Input: dimensioned drawing with shaded views. Units: mm. Origin: part minimum x, y, z. A direction names the side the tool comes from. Coordinates: 2 decimals unless noted, no trailing zeros. Order: outer loops, then holes, each group sorted by start corner. A loop starts at its lowest first (then second) coordinate and runs counter-clockwise, first axis right, second up.
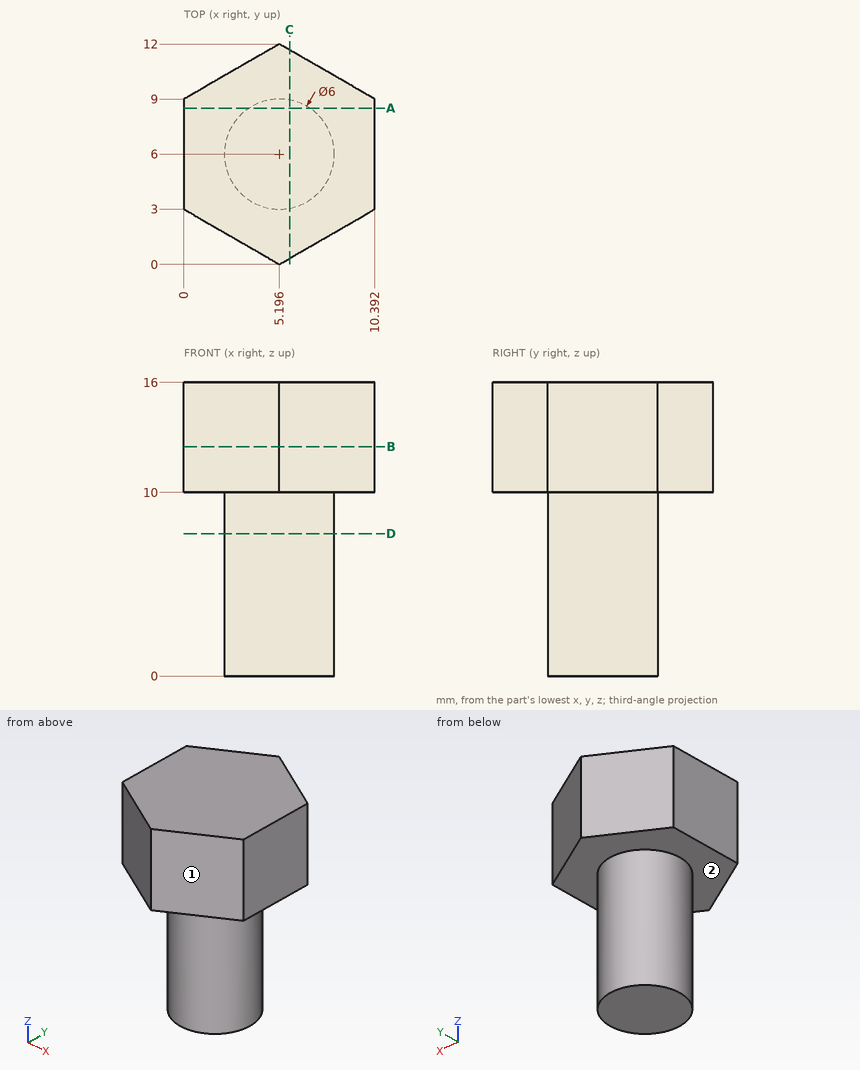
1. Contact query for flat-ended pins moving along their axis: P1, Ø5, axis at x = 9, z = 13.5, coming from the +Y side; P2, Ø4, axis at x = 2.5, z = 7.5, coming from the +Y side. Output: stop coordinate, or through.
2. Section query C-C, the plane x = 5.75. Output: boundary loops of the cut face in (y, z).
3. Access query for the marked faces 1 and 2. Directions: +Z, -Z, +X, -X, +Y, -Y. A direction counts if a zero-diameter tool reaches every point of the face in a straight line with its end or side. Return the directions, or none.
4. Section query D-D, the plane z = 7.75. Output: boundary loops of the cut face in (x, y), plus the area to 3 significant figures.
5. Material intervals for line 1 along Z through (x, y) = (10.25, 5.25); line 2 along Y through (x, z) = (7.5, 0.5); line 3 along Y through (x, z) = (4.25, 5.25), sorted ascending.
6. Section query B-B, the plane z = 12.5. Output: boundary loops of the cut face in (x, y).
7. Section query A-A, the plane y = 8.5. Output: boundary loops of the cut face in (x, z) (1 decimal).
Answer key:
1. P1: stops at y = 11.25
1. P2: stops at y = 8.92
2. outline: (0.32, 10) - (3.05, 10) - (3.05, 0) - (8.95, 0) - (8.95, 10) - (11.68, 10) - (11.68, 16) - (0.32, 16) - close
3. face 1: +Z, -Z, +X, -Y
3. face 2: -Z
4. outline: circle Ø6 at (5.2, 6)
4. area: 28.3 mm2
5. line 1: z = 10 to 16
5. line 2: y = 4.08 to 7.92
5. line 3: y = 3.15 to 8.85
6. outline: (0, 3) - (5.2, 0) - (10.39, 3) - (10.39, 9) - (5.2, 12) - (0, 9) - close
7. outline: (0, 10) - (3.5, 10) - (3.5, 0) - (6.9, 0) - (6.9, 10) - (10.4, 10) - (10.4, 16) - (0, 16) - close
